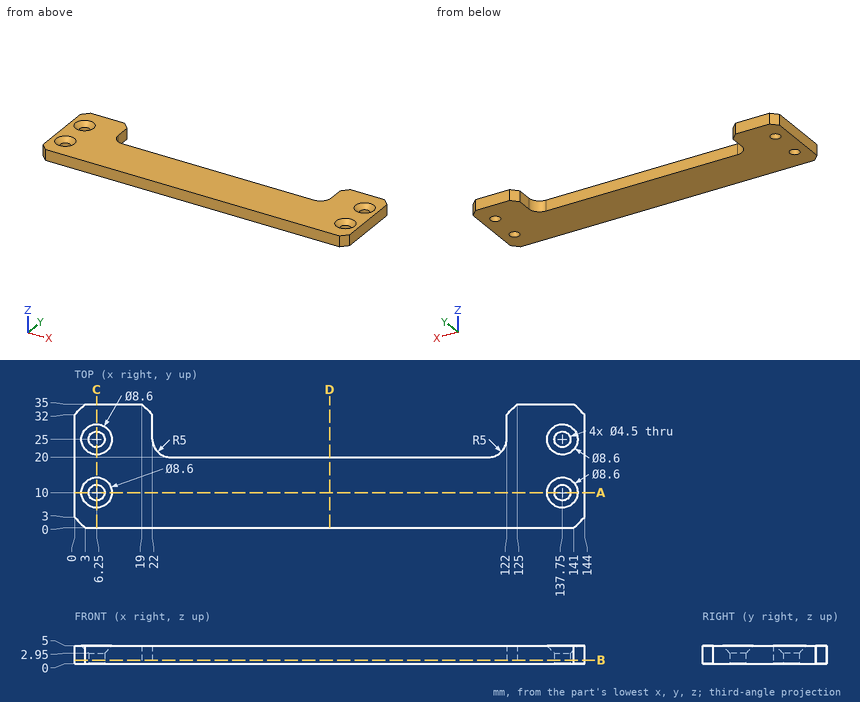
Print and shaded views of the part. All mm, measured from the part's lowest x, y and z. Give positions to 0.01 mm unless a question says otherwise; leave off trailing zeros. Write each loop counter-clockwise with the first axis right and the second up, starting at its lowest first coordinate (ties: lowest second). Pieces come first, ordered by that corner, then holes. Notation, with made-up numbers: M 34.5,-30 L 87.5,-30 A14 ccw 87.5,-11 Z; hole C -35.75,38 d1. An arc over 180 degrees is marked long. Use a Markdown table: item, result.
1) Drill centre lines: line 1 (Y direction, x = 6.25, z = 1.8); line 2 (X direction, y = 25, z = 0.7); line 3 (X direction, y = 10, z = 0.65). Where is each one in solid material? Low to high. Write a range as from..to.
Responses:
| item | result |
|---|---|
| line 1 | y = 0..7.75, 12.25..22.75, 27.25..35 |
| line 2 | x = 0..4, 8.5..22, 122..135.5, 140..144 |
| line 3 | x = 0..4, 8.5..135.5, 140..144 |
2) Cut at D-D (x = 72). List the corners of the cut face in (y, z).
Responses:
| item | result |
|---|---|
| outline | M 0,0 L 20,0 L 20,5 L 0,5 Z |
3) Cut at C-C (x = 6.25). List the corners of the cut face in (y, z).
Responses:
| item | result |
|---|---|
| outline | M 0,0 L 7.75,0 L 7.75,2.95 L 5.7,5 L 0,5 Z; M 12.25,0 L 22.75,0 L 22.75,2.95 L 20.7,5 L 14.3,5 L 12.25,2.95 Z; M 27.25,0 L 35,0 L 35,5 L 29.3,5 L 27.25,2.95 Z |
4) Pin check, flat tips, straight feed: pin 1 (3 mm diameter, centred on x = 122, y = 17.5, fed in from -Z); pin 2 (1.5 mm diameter, centred on x = 81.5, z = 3.5, fed in from +Y); pin 3 (6 mm diameter, centred on x = 137.75, y = 25, fed in from +Z). Stop position of each tip, or through.
Responses:
| item | result |
|---|---|
| pin 1 | stops at z = 0 |
| pin 2 | stops at y = 20 |
| pin 3 | stops at z = 3.7 |
5) Cut at A-A (y = 10). List the corners of the cut face in (x, z), and give its area (3 significant figures).
Responses:
| item | result |
|---|---|
| outline | M 0,0 L 4,0 L 4,2.95 L 1.95,5 L 0,5 Z; M 8.5,0 L 135.5,0 L 135.5,2.95 L 133.45,5 L 10.55,5 L 8.5,2.95 Z; M 140,0 L 144,0 L 144,5 L 142.05,5 L 140,2.95 Z |
| area | 667 mm2 |
6) Cut at B-B (z = 1). List the corners of the cut face in (x, y).
Responses:
| item | result |
|---|---|
| outline | M 0,3 L 3,0 L 141,0 L 144,3 L 144,32 L 141,35 L 125,35 L 122,32 L 122,25 A5 cw 117,20 L 27,20 A5 cw 22,25 L 22,32 L 19,35 L 3,35 L 0,32 Z; hole C 6.25,10 d4.5; hole C 6.25,25 d4.5; hole C 137.75,10 d4.5; hole C 137.75,25 d4.5 |
